Geometry check sheet. Reference: the model listing, model coordinates, mm. Face numbers are marked on the shaded views. Round coordinates to 2 decimals unless told otherwise and drop trailing zeros. Order: outer loops, then holes, each group sorted by start corner. A loop starts at its lowest first (then second) coordinate and runs counter-clockwise, first axis right, second up.
(1) Material ranges on line 1 along Y through (x, z) = (0, 5.5); line 2 along X through (y, z) = (-2, 8); line 3 along X through (y, z) = (-3.5, 1.75), recorded low to high.
(2) Sectioned sample at D-D (x = 11.25). Record the boundary of the cut face in (y, z).
(3) Release check for a two-part mould opening along Y. For the marked faces 1, 2, 3 and 4 record: +Y half, -Y half, draft (parallel to the pull), parting line (faces both ways), or undercut.
(4) Sectioned sample at B-B (x = -2.5). Record the boundary of the cut face in (y, z), plus the area to 4 significant figures.
(5) Go/stop test with a flat-tipped pin: pin 1 (6.5 mm diameter, centred on x = 0, y = 0, fed in from -Z). Record where the tip stops, or that it passes through.
(6) Sectioned sample at A-A (y = 0). Record the boundary of the cut face in (x, z).
(7) Sectioned sample at C-C (z = 8.75). Record the boundary of the cut face in (x, y), plus the area to 3 significant figures.
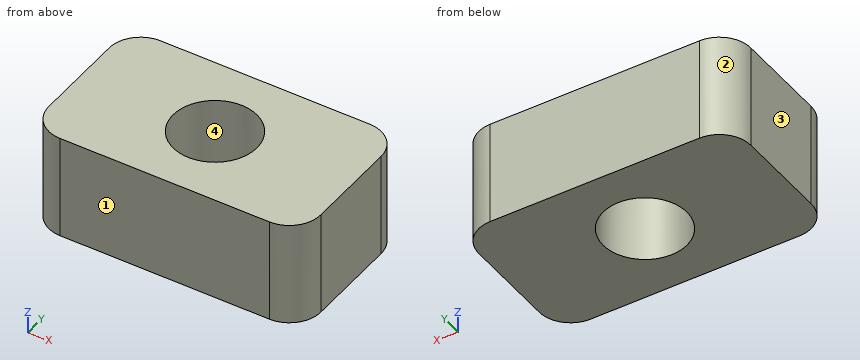
from build123d import *

# Parameters (mm, degrees)
SKETCH1_W           = 26
SKETCH1_H           = 15
SKETCH1_R           = 4
BOSS_EXTRUDE1_DEPTH = 10
FILLET1_R           = 3


with BuildPart() as part:
    # Sketch1 → Boss-Extrude1 (new body)
    with BuildSketch(Plane.XY):
        Rectangle(SKETCH1_W, SKETCH1_H)
        Circle(SKETCH1_R, mode=Mode.SUBTRACT)
    extrude(amount=BOSS_EXTRUDE1_DEPTH)

    # Fillet1
    fillet1_edges = [part.edges().sort_by_distance(p)[0] for p in [
        (13, -7.5, 5),
        (-13, -7.5, 5),
        (-13, 7.5, 5),
        (13, 7.5, 5),
    ]]
    fillet(fillet1_edges, radius=FILLET1_R)


solid = part.part
Answer below:
1. line 1: y = -7.5 to -4, 4 to 7.5
1. line 2: x = -13 to -3.46, 3.46 to 13
1. line 3: x = -13 to -1.94, 1.94 to 13
2. outline: (-7.23, 0) - (7.23, 0) - (7.23, 10) - (-7.23, 10) - close
3. face 1: -Y half
3. face 2: +Y half
3. face 3: draft
3. face 4: undercut
4. outline: (-7.5, 0) - (-3.12, 0) - (-3.12, 10) - (-7.5, 10) - close; (3.12, 0) - (7.5, 0) - (7.5, 10) - (3.12, 10) - close
4. area: 87.55 mm2
5. pin 1: passes through
6. outline: (-13, 0) - (-4, 0) - (-4, 10) - (-13, 10) - close; (4, 0) - (13, 0) - (13, 10) - (4, 10) - close
7. outline: (-13, -4.5) arc R3 ccw to (-10, -7.5) - (10, -7.5) arc R3 ccw to (13, -4.5) - (13, 4.5) arc R3 ccw to (10, 7.5) - (-10, 7.5) arc R3 ccw to (-13, 4.5) - close; hole circle Ø8 at (0, 0)
7. area: 332 mm2
